Geometry: final body of the model. Coordinates: model frame, mm. A direction names the side the tool comes from. Round coordinates to 2 decimals unless told otherwise and drop trailing zeros. Write each loop counter-clockwise with the first axis right and the second up, starting at its lowest first coordinate (ties: lowest second). Pieces come first, ordered by that corner, then holes. Notation, with made-up numbers: (21, -7) -> (67, -7) arc R18 cw to (67, 15) -> close; hole circle Ø10 at (-4.5, 74). An arc over 180 degrees is marked (long way). One line per item, written item: value. Start each with the question number.
from build123d import *

# Parameters (mm, degrees)
TORSO_BLOCK_DEPTH        = 8
TORSO_SHELL_1MM_T        = -1
NECK_STUD_SKETCH_R       = 2
NECK_STUD_4_DEPTH        = 5
ARM_HOLE_1_3_REACH       = 23.606
ARM_HOLE_1_SKETCH_R      = 2
ARM_HOLE_2_3_REACH       = 26.042
ARM_HOLE_2_SKETCH_R      = 2
HIP_CONNECTOR_SKETCH_W   = 3
HIP_CONNECTOR_SKETCH_H   = 6
HIP_CONNECTOR_BOSS_DEPTH = 5


with BuildPart() as part:
    # Torso Profile Sketch → Torso Block (new body)
    with BuildSketch(Plane.XY):
        Polygon((0, 0), (15, 0), (12.5, 12), (2.5, 12), align=None)
    extrude(amount=-TORSO_BLOCK_DEPTH)

    # Torso Shell 1mm
    torso_shell_1mm_openings = [part.faces().sort_by_distance(p)[0] for p in [
        (7.5, 0, -4),
    ]]
    offset(amount=TORSO_SHELL_1MM_T, openings=torso_shell_1mm_openings, kind=Kind.INTERSECTION)

    # Neck Stud Sketch → Neck Stud Ø4 (add)
    with BuildSketch(Plane(origin=(0, 12, 0), x_dir=(1, 0, 0), z_dir=(0, 1, 0))):
        with Locations(Location((7.5, 4, 0), (0, 0, 270))):
            Circle(NECK_STUD_SKETCH_R)
    extrude(amount=NECK_STUD_4_DEPTH)

    # Arm Hole 1 Sketch → Arm Hole 1 Ø3 (cut, up to next)
    with BuildSketch(Plane(origin=(14.376039933, 2.995008319, 0), x_dir=(0, 0, -1), z_dir=(0.978980419737605, 0.20395425411200113, 0)), mode=Mode.PRIVATE) as arm_hole_1_3_sk1:
        with Locations(Location((4, 6.940686188, 0), (0, 0, 90))):
            Circle(ARM_HOLE_1_SKETCH_R)
    arm_hole_1_3_tool1 = extrude(arm_hole_1_3_sk1.sketch, amount=-ARM_HOLE_1_3_REACH, mode=Mode.PRIVATE) & part.part
    add(arm_hole_1_3_tool1.solids().sort_by_distance((12.960457, 9.789804, -4))[0], mode=Mode.SUBTRACT)

    # Arm Hole 2 Sketch → Arm Hole 2 Ø3 (cut, up to next)
    with BuildSketch(Plane(origin=(0, 0, 0), x_dir=(0, 0, 1), z_dir=(-0.978980419737605, 0.20395425411200113, 0)), mode=Mode.PRIVATE) as arm_hole_2_3_sk1:
        with Locations(Location((-4, 10, 0), (0, 0, 270))):
            Circle(ARM_HOLE_2_SKETCH_R)
    arm_hole_2_3_tool1 = extrude(arm_hole_2_3_sk1.sketch, amount=-ARM_HOLE_2_3_REACH, mode=Mode.PRIVATE) & part.part
    add(arm_hole_2_3_tool1.solids().sort_by_distance((2.039543, 9.789804, -4))[0], mode=Mode.SUBTRACT)

    # Hip Connector Sketch → Hip Connector Boss (add)
    with BuildSketch(Plane.XZ):
        with Locations((7.5, -4)):
            Rectangle(HIP_CONNECTOR_SKETCH_W, HIP_CONNECTOR_SKETCH_H)
    extrude(amount=-HIP_CONNECTOR_BOSS_DEPTH)


solid = part.part
(1) Set-up query: faces 1 (the face through (6, 2, -4)), 2 (the face through (7, 6, -1)), 3 (the face through (8.852, 14.465, -5.474)). Return all of +Z, -Z, +X, -X, +Y, -Y with unobstructed straight access to the full face (end or side cutting, diameter ignored); none if empty.
(2) Section query A-A (x = 7.5). Output: boundary loops of the cut face in (y, z).
(3) Pin query (flat end, axial travel): pin 1 (1.5 mm diameter, centred on y = 10, z = -7, fed in from -X); pin 2 (2.5 mm diameter, centred on y = 2.5, z = -3.5, fed in from +X); pin 3 (4 mm diameter, centred on x = 3.5, z = -6, fed in from +Y). Return the tip coordinate at first contact, or that it passes through.
(4) Section query B-B (z = -4). Output: boundary loops of the cut face in (x, y), and give its area (3 significant figures).
(5) Section query C-C (y = 15). Output: boundary loops of the cut face in (x, z).
(6) Line query: probe 1 along X at (y, z) = (4, -2.25); probe 2 along Z at (x, y) = (5.75, 5.75); probe 3 along X at (y, z) = (1.75, -5). Output: solid intervals per line, ascending.
(7) Pull-direction query (X, two-part tool) for faces 4 (the face through (7, 0, -4)), 5 (the face through (13.768, 5.916, -3.944)), 6 (the face through (1.929, 4.355, -3.958)); classes: pulls with the +X half, pulls with the -X half, needs draft (parallel to the pull), parting line crosses it, or undercut.
Results list:
1. face 1: -Y
1. face 2: none
1. face 3: +Y
2. outline: (0, -8) -> (12, -8) -> (12, -6) -> (17, -6) -> (17, -2) -> (12, -2) -> (12, 0) -> (0, 0) -> close; hole (5, -7) -> (11, -7) -> (11, -1) -> (5, -1) -> close
3. pin 1: stops at x = 1.93
3. pin 2: stops at x = 14.74
3. pin 3: stops at y = 12
4. outline: (0, 0) -> (1.02, 0) -> (2.61, 7.63) -> (1.63, 7.83) -> close; (2.45, 11.75) -> (6.04, 11) -> (8.96, 11) -> (12.55, 11.75) -> (12.5, 12) -> (9.5, 12) -> (9.5, 17) -> (5.5, 17) -> (5.5, 12) -> (2.5, 12) -> close; (6, 0) -> (9, 0) -> (9, 5) -> (6, 5) -> close; (12.39, 7.63) -> (13.98, 0) -> (15, 0) -> (13.37, 7.83) -> close
4. area: 58.2 mm^2
5. outline: circle Ø4 at (7.5, -4)
6. probe 1: x = 0.83 to 1.85, 6 to 9, 13.15 to 14.17
6. probe 2: z = -8 to -7, -1 to 0
6. probe 3: x = 0.36 to 1.39, 6 to 9, 13.61 to 14.64
7. face 4: needs draft
7. face 5: pulls with the +X half
7. face 6: undercut
